```python
from build123d import *

# Parameters (mm, degrees)
SKETCH1_R                = 45
BOSS_EXTRUDE1_DEPTH      = 240
BOSS_EXTRUDE2_DEPTH      = 76
BOSS_EXTRUDE2_DEPTH_BACK = 76
SKETCH2_R                = 100
CHAMFER1_SIZE            = 6


with BuildPart() as part:
    # Sketch1 → Boss-Extrude1 (new body)
    with BuildSketch(Plane(origin=(0, 0, 0), x_dir=(1, 0, 0), z_dir=(0, 1, 0))):
        with Locations(Location((0, 0, 0), (0, 0, 270))):
            Circle(SKETCH1_R)
    extrude(amount=BOSS_EXTRUDE1_DEPTH)

    # Sketch2 → Boss-Extrude2 (add, two sides: drawn at the far end of the back side and taken through both)
    with BuildSketch(Plane(origin=(0, 120, 0), x_dir=(1, 0, 0), z_dir=(0, 1, 0)).offset(-BOSS_EXTRUDE2_DEPTH_BACK)):
        with Locations(Location((0, 0, 0), (0, 0, 270))):
            Circle(SKETCH2_R)
    extrude(amount=BOSS_EXTRUDE2_DEPTH + BOSS_EXTRUDE2_DEPTH_BACK)

    # Chamfer1
    chamfer1_edges = [part.edges().sort_by_distance(p)[0] for p in [
        (0, 44, -100),
        (0, 196, -100),
    ]]
    chamfer(chamfer1_edges, length=CHAMFER1_SIZE)


solid = part.part
```
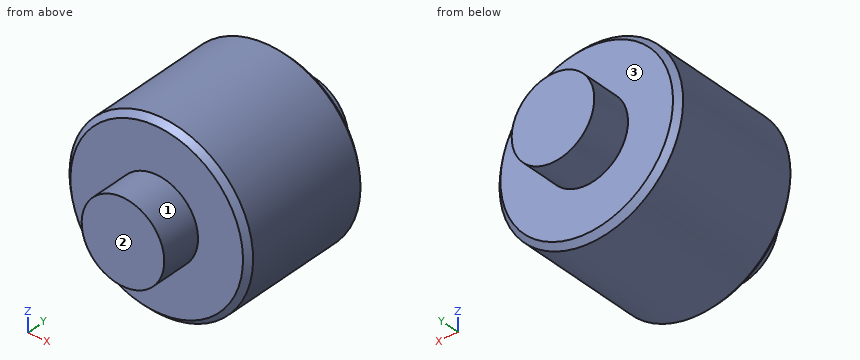
The listing builds one solid part. Answer for the finished solid, in the listing's coordinates (mm). Face numbers are marked on the shaded views. A direction names the side the tool comes from. Coordinates: 2 decimals unless noted, no trailing zeros. Loops run counter-clockwise (first coordinate to the right, second up) from the corner with the lowest first, then second, coordinate; pieces in that order, holes last. Notation, with made-up numbers: (-25, 12) - (-17, 12) arc R35 cw to (-17, 51) - close; hole circle Ø10 at (32, 89.5). An arc over 180 degrees is marked (long way). Use a Markdown table: item, result. Add a question column.
1) The part is cut by section C-C, the plane y = 87. Give the vertices of the cut face in (x, z).
2) The part is cut by section A-A, the plane z = 0. Give the vertices of the cut face in (x, y), and give its area (3 significant figures).
3) Find the intervals of material crossed by line 1 (Y direction, x = 49, z = 15.5); line 2 (X direction, y = 109, z = -30); line 3 (X direction, y = 127.5, z = 33.5), in increasing order.
4) The part is cut by section B-B, the plane x = 0. Give the vertices of the cut face in (y, z).
5) For the marked faces 1, 2 and 3, determine the directions among +Z, -Z, +X, -X, +Y, -Y from which every point of the face is accessible in a straight line to the end or side of a thin tool.
6) Given pin 1 (2 mm diameter, centred on x = -67.5, z = 7, fed in from -Y); pin 2 (5 mm diameter, centred on y = 85.5, z = -71, fed in from -X); pin 3 (6 mm diameter, centred on y = 77.5, z = 37.5, fed in from -X), each flat-ended and moving along its own axis, determine where each tip first touches the part or whether it passes through.
Here are the results:
| question | item | result |
|---|---|---|
| 1 | outline | circle Ø200 at (0, 0) |
| 2 | outline | (-100, 50) - (-94, 44) - (-45, 44) - (-45, 0) - (45, 0) - (45, 44) - (94, 44) - (100, 50) - (100, 190) - (94, 196) - (45, 196) - (45, 240) - (-45, 240) - (-45, 196) - (-94, 196) - (-100, 190) - close |
| 2 | area | 38,200 mm^2 |
| 3 | line 1 | y = 44 to 196 |
| 3 | line 2 | x = -95.39 to 95.39 |
| 3 | line 3 | x = -94.22 to 94.22 |
| 4 | outline | (0, -45) - (44, -45) - (44, -94) - (50, -100) - (190, -100) - (196, -94) - (196, -45) - (240, -45) - (240, 45) - (196, 45) - (196, 94) - (190, 100) - (50, 100) - (44, 94) - (44, 45) - (0, 45) - close |
| 5 | face 1 | -Y |
| 5 | face 2 | +Z, -Z, +X, -X, -Y |
| 5 | face 3 | +Y |
| 6 | pin 1 | stops at y = 44 |
| 6 | pin 2 | stops at x = -72.85 |
| 6 | pin 3 | stops at x = -93.86 |
